```python
from build123d import *

# Parameters (mm, degrees)
SKETCH1_R           = 4
BOSS_EXTRUDE1_DEPTH = 6


with BuildPart() as part:
    # Sketch1 → Boss-Extrude1 (new body)
    # profile 1 of 5: a face of its own
    with BuildSketch(Plane(origin=(0, 0, 0), x_dir=(0, 0, -1), z_dir=(1, 0, 0))):
        with BuildLine():
            Line((38.416871989, -99.116819696), (65.778483455, -23.941410033))
            ThreePointArc((65.778483455, -23.941410033), (60.607739865, -29.58428647), (52.961355814, -29.918134807))
            Line((52.961355814, -29.918134807), (43.564429606, -26.497933374))
            Line((43.564429606, -26.497933374), (19.623019573, -92.276416829))
            ThreePointArc((19.623019573, -92.276416829), (25.599744348, -105.09354447), (38.416871989, -99.116819696))
        make_face()
        with Locations((29.019945781, -95.696618262)):
            Circle(SKETCH1_R, mode=Mode.SUBTRACT)
    # profile 2 of 5: a face of its own
    with BuildSketch(Plane(origin=(0, 0, 0), x_dir=(0, 0, -1), z_dir=(1, 0, 0))):
        with BuildLine():
            ThreePointArc((65.778483455, -23.941410033), (65.444635118, -16.295025982), (59.80175868, -11.124282392))
            ThreePointArc((59.80175868, -11.124282392), (52.15537463, -11.458130729), (46.984631039, -17.101007166))
            Line((46.984631039, -17.101007166), (43.564429606, -26.497933374))
            Line((43.564429606, -26.497933374), (52.961355814, -29.918134807))
            ThreePointArc((52.961355814, -29.918134807), (60.607739865, -29.58428647), (65.778483455, -23.941410033))
        make_face()
        with Locations((56.381557247, -20.5212086)):
            Circle(SKETCH1_R, mode=Mode.SUBTRACT)
    # profile 3 of 5: a face of its own
    with BuildSketch(Plane(origin=(0, 0, 0), x_dir=(0, 0, -1), z_dir=(1, 0, 0))):
        with BuildLine():
            Line((59.80175868, -11.124282392), (10, 7.002075382))
            Line((10, 7.002075382), (10, 0))
            ThreePointArc((10, 0), (5.735764364, -8.191520443), (-3.420201433, -9.396926208))
            Line((-3.420201433, -9.396926208), (43.564429606, -26.497933374))
            Line((43.564429606, -26.497933374), (46.984631039, -17.101007166))
            ThreePointArc((46.984631039, -17.101007166), (52.15537463, -11.458130729), (59.80175868, -11.124282392))
        make_face()
    # profile 4 of 5: a face of its own
    with BuildSketch(Plane(origin=(0, 0, 0), x_dir=(0, 0, -1), z_dir=(1, 0, 0))):
        with BuildLine():
            Line((10, 0), (10, 7.002075382))
            Line((10, 7.002075382), (3.420201433, 9.396926208))
            ThreePointArc((3.420201433, 9.396926208), (-5.735764364, 8.191520443), (-10, 0))
            ThreePointArc((-10, 0), (-8.191520443, -5.735764364), (-3.420201433, -9.396926208))
            ThreePointArc((-3.420201433, -9.396926208), (5.735764364, -8.191520443), (10, 0))
        make_face()
        Circle(SKETCH1_R, mode=Mode.SUBTRACT)
    # profile 5 of 5: a face of its own
    with BuildSketch(Plane(origin=(0, 0, 0), x_dir=(0, 0, -1), z_dir=(1, 0, 0))):
        with BuildLine():
            Line((10, 7.002075382), (10, 80))
            ThreePointArc((10, 80), (0, 90), (-10, 80))
            Line((-10, 80), (-10, 0))
            ThreePointArc((-10, 0), (-5.735764364, 8.191520443), (3.420201433, 9.396926208))
            Line((3.420201433, 9.396926208), (10, 7.002075382))
        make_face()
        with Locations((0, 80)):
            Circle(SKETCH1_R, mode=Mode.SUBTRACT)
    extrude(amount=BOSS_EXTRUDE1_DEPTH)


solid = part.part
```
The model under review builds one solid part; all positions refer to its coordinate system, in mm. A direction names the side the tool comes from. Give positions to 0.01 mm unless a question says otherwise; leave off trailing zeros. Write each loop counter-clockwise with the first axis right and the second up, starting at its lowest first coordinate (ties: lowest second). Pieces come first, ordered by that corner, then holes. Notation, with made-up numbers: (51, -20.5) -> (110, -20.5) arc R25 ccw to (110, -2.5) -> close; hole circle Ø10 at (-36.75, 2.5). An arc over 180 degrees is marked (long way). Put each result on its own line as item: value.
(1) Tool access review of faces 5 (the flat face through (2.958, -17.828, -19.743)), 6 (the cylindrical face through (2.96, -16.39, -65.49)), 7 (the flat face through (3, 43, -10)): name each direction out of +Z, -Z, +X, -X, +Y, -Y from which nothing blocks a thin tool from reaching the whole face with its end or side.
Results are:
face 5: +Z, +X, -X
face 6: -Z, +X, -X
face 7: -Z, +X, -X, +Y
(2) We need section B-B, the plane x = 3. Give the boundary of the cut face in (y, z).
Results are:
outline: (-99.12, -38.42) -> (-23.94, -65.78) arc R10 ccw to (-11.12, -59.8) -> (7, -10) -> (80, -10) arc R10 ccw to (80, 10) -> (0, 10) arc R10 ccw to (-9.4, 3.42) -> (-26.5, -43.56) -> (-92.28, -19.62) arc R10 ccw to start; hole circle Ø8 at (-95.7, -29.02); hole circle Ø8 at (-20.52, -56.38); hole circle Ø8 at (0, 0); hole circle Ø8 at (80, 0)
(3) The part is to be moulded in two halves that separate along Z. For faces 1 (the cylindrical face through (2.958, -99.245, -30.866)), 2 (the flat face through (2.96, -58.93, -31.76)), 3 (the flat face through (0, -7, -22)), 4 (the cylindrical face through (2.958, -3.905, 0.867)), say which applies: pulls with the +Z half, pulls with the -Z half, needs draft (parallel to the pull), parting line crosses it, or undercut.
Results are:
face 1: undercut
face 2: pulls with the +Z half
face 3: needs draft
face 4: undercut
(4) For pin 1 Ø1 at (x, y) = (3.5, -30) entering from -Z; pin 2 Ø1.5 at (y, z) = (1, 2) entering from +X; pin 3 Ø1 at (x, z) = (1, -23.5) entering from -Y, all flat-tipped, find the tip position at first contact; note any pin that passes through.
Results are:
pin 1: z = -63.76
pin 2: through
pin 3: y = -104.35
(5) We need section D-D, the plane z = -50. Give the boundary of the cut face in (x, y).
Results are:
outline: (0, -67.29) -> (6, -67.29) -> (6, -7.56) -> (0, -7.56) -> close
(6) To check wall thickness, follow probe 1 along Y at (x, z) = (2.8, 0); probe 2 along Z at (x, y) = (1.85, 28); probe 3 along Y at (x, z) = (4.9, -16.5). State the ranges of each line that lie inside material, in increasing order. Write a range as from..to.
Results are:
probe 1: -10.64..-4, 4..76, 84..90
probe 2: -10..10
probe 3: -16.65..4.64
(7) We need section C-C, the plane y = -6. Give the boundary of the cut face in (x, z).
Results are:
outline: (0, -45.72) -> (6, -45.72) -> (6, 8) -> (0, 8) -> close
(8) We need section A-A, the plane z = 0. Give the boundary of the cut face in (x, y).
Results are:
outline: (0, -10.64) -> (6, -10.64) -> (6, -4) -> (0, -4) -> close; (0, 4) -> (6, 4) -> (6, 76) -> (0, 76) -> close; (0, 84) -> (6, 84) -> (6, 90) -> (0, 90) -> close
